```python
from build123d import *

# Parameters (mm, degrees)
SKETCH1_W               = 15
SKETCH1_H               = 15
BOSS_EXTRUDE1_DEPTH     = 25
CUT_EXTRUDE1_DEPTH      = 31.103986447
CUT_EXTRUDE1_DEPTH_BACK = 31.103986447
SKETCH2_R               = 3


with BuildPart() as part:
    # Sketch1 → Boss-Extrude1 (new body)
    with BuildSketch(Plane.XY):
        Rectangle(SKETCH1_W, SKETCH1_H)
    extrude(amount=BOSS_EXTRUDE1_DEPTH)

    # Sketch2 → Cut-Extrude1 (cut, two sides: drawn at the far end of the back side and taken through both)
    with BuildSketch(Plane.ZY.offset(7.5).offset(-CUT_EXTRUDE1_DEPTH_BACK)):
        with Locations((17, 0)):
            Circle(SKETCH2_R)
    extrude(amount=CUT_EXTRUDE1_DEPTH + CUT_EXTRUDE1_DEPTH_BACK, mode=Mode.SUBTRACT)


solid = part.part
```
The listing builds one solid part. Answer for the finished solid, in the listing's coordinates (mm). Coordinates: 2 decimals unless noted, no trailing zeros. Write each loop counter-clockwise with the first axis right and the second up, starting at its lowest first coordinate (ties: lowest second). Pieces come first, ordered by that corner, then holes. Notation, with made-up numbers: (22, 84.5) - (60, 84.5) arc R14 ccw to (60, 90.5) - close; hole circle Ø2 at (-30, -13.75). An arc over 180 degrees is marked (long way). One line per item, written item: value.
1) Find section B-B (z = 17). Give the vertices of the cut face in (x, y), and give its area (3 significant figures).
Geometry check:
outline: (-7.5, -7.5) - (7.5, -7.5) - (7.5, -3) - (-7.5, -3) - close; (-7.5, 3) - (7.5, 3) - (7.5, 7.5) - (-7.5, 7.5) - close
area: 135 mm2
2) Consider line 1 along Y through (x, z) = (-4.25, 17); line 2 along Z through (x, y) = (0.75, 0); line 3 along Z through (x, y) = (2.5, 1.5). Determine where each line is inside the solid, lowest interval first. Write a range as from..to.
Geometry check:
line 1: y = -7.5..-3, 3..7.5
line 2: z = 0..14, 20..25
line 3: z = 0..14.4, 19.6..25
3) Find section C-C (x = -2). Give the vertices of the cut face in (y, z), and give its area (3 significant figures).
Geometry check:
outline: (-7.5, 0) - (7.5, 0) - (7.5, 25) - (-7.5, 25) - close; hole circle Ø6 at (0, 17)
area: 347 mm2
4) Find section A-A (y = 0). Give the vertices of the cut face in (x, z), and give its area (3 significant figures).
Geometry check:
outline: (-7.5, 0) - (7.5, 0) - (7.5, 14) - (-7.5, 14) - close; (-7.5, 20) - (7.5, 20) - (7.5, 25) - (-7.5, 25) - close
area: 285 mm2
5) For a pull along Z with two mould halves and no side action, classify faces 1 (the flat face through (-7.5, 0, 12)), 2 (the cylindrical face through (0.1, -1.8, 14.6)), 3 (the flat face through (0, 0, 0)) as pulls with the +Z half, pulls with the -Z half, needs draft (parallel to the pull), parting line crosses it, or undercut.
Geometry check:
face 1: needs draft
face 2: undercut
face 3: pulls with the -Z half
